```python
from build123d import *

# Parameters (mm, degrees)
SKETCH_1_W              = 200
SKETCH_1_H              = 120
EXTRUDE_1_DEPTH         = 20
HOLE_WIZARD_15_0_15_1_D = 15
CHAMFER_1_SIZE          = 5


with BuildPart() as part:
    # 草图1 → 凸台-拉伸1 (new body)
    with BuildSketch(Plane(origin=(0, 0, 0), x_dir=(0, 0, -1), z_dir=(1, 0, 0))):
        Rectangle(SKETCH_1_W, SKETCH_1_H)
    extrude(amount=EXTRUDE_1_DEPTH)

    # Ø15.0 (15) 直径孔1 (through all)
    with Locations(Plane(origin=(20, 0, 0), x_dir=(0, 0, -1), z_dir=(1, 0, 0))):
        with Locations((-75, 0), (75, 0)):
            Hole(HOLE_WIZARD_15_0_15_1_D / 2)

    # 倒角1
    chamfer_1_edges = [part.edges().sort_by_distance(p)[0] for p in [
        (10, -60, -100),
        (10, -60, 100),
        (10, 60, 100),
        (10, 60, -100),
    ]]
    chamfer(chamfer_1_edges, length=CHAMFER_1_SIZE)


solid = part.part
```
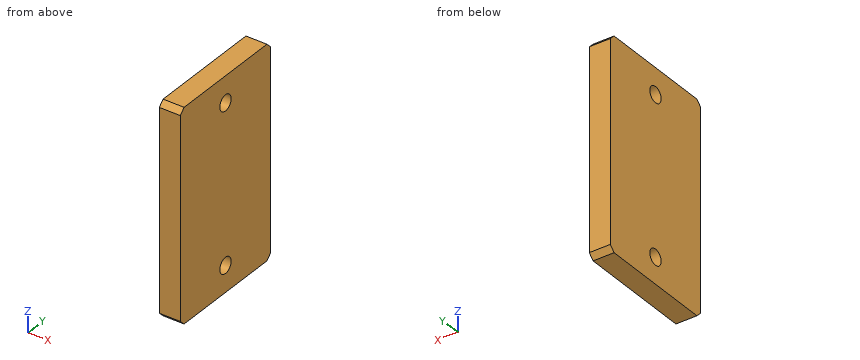
CAD build for the part. Positions are in the model's coordinates, mm. Round coordinates to 2 decimals unless told otherwise and drop trailing zeros. Order: outer loops, then holes, each group sorted by start corner. A loop starts at its lowest first (then second) coordinate and runs counter-clockwise, first axis right, second up.
Q1. Drop a flat-ended pin along its axis: pin 1 (1 mm diameter, centred on y = -17, z = 12, fed in from -X). Give the stop position or say it passes through.
Q2. Slice it at D-D (z = -78.5). Write the cut outline in (x, y).
Q3. Slice it at A-A (y = 0). Write the cut outline in (x, z), and give its area (3 significant figures).
Q4. Wall check: L1, parallel to Y at x = 15.75, z = 75.5; L2, parallel to Y at x = 17.5, z = 74. Give the ranges that are in metal, low to high.
Q5. Slice it at C-C (x = 9.25). Write the cut outline in (y, z), and give its area (3 significant figures).
Q6. Slice it at B-B (z = 75). Write the cut outline in (x, y).
Results below:
1. pin 1: stops at x = 0
2. outline: (0, -60) - (20, -60) - (20, -6.63) - (0, -6.63) - close; (0, 6.63) - (20, 6.63) - (20, 60) - (0, 60) - close
3. outline: (0, -100) - (20, -100) - (20, -82.5) - (0, -82.5) - close; (0, -67.5) - (20, -67.5) - (20, 67.5) - (0, 67.5) - close; (0, 82.5) - (20, 82.5) - (20, 100) - (0, 100) - close
3. area: 3,400 mm2
4. L1: y = -60 to -7.48, 7.48 to 60
4. L2: y = -60 to -7.43, 7.43 to 60
5. outline: (-60, -95) - (-55, -100) - (55, -100) - (60, -95) - (60, 95) - (55, 100) - (-55, 100) - (-60, 95) - close; hole circle Ø15 at (0, -75); hole circle Ø15 at (0, 75)
5. area: 23,600 mm2
6. outline: (0, -60) - (20, -60) - (20, -7.5) - (0, -7.5) - close; (0, 7.5) - (20, 7.5) - (20, 60) - (0, 60) - close
